Print and shaded views of the part. All mm, measured from the part's lowest x, y and z. Coordinates: 2 decimals unless noted, no trailing zeros. Order: outer loops, then holes, each group sorted by start corner. A loop starts at its lowest first (then second) coordinate and runs counter-clockwise, first axis right, second up. Notation, with made-up numbers: (22, -17) -> (54, -17) arc R26 ccw to (54, 20) -> close; hole circle Ø10 at (70.5, -2.75). An arc over 180 degrees is marked (long way). Write item = value, one per line. Start each with the question number.
Q1. Mould opens along Y. For the marked faces 1 and 2 say: +Y half, -Y half, draft (parallel to the pull), parting line (faces both ways), or undercut.
Q2. Flat gauge pins, fed straight in: pin 1 (8.5 mm diameter, centred on x = 82, y = 39, fed in from +Z); pin 2 (1.5 mm diameter, centred on y = 69.5, z = 6, fed in from -X) (1 decimal); pin 3 (4 mm diameter, centred on x = 81.5, z = 4.5, fed in from +Y); pin 4 (5 mm diameter, centred on x = 37, z = 4, fed in from -Y) (1 decimal). Where does each tip first touch, or does it go through?
Q3. Cut at B-B, the plane z = 1.75. List the corners of the cut face in (x, y), plus the area to 3 significant figures.
Q4. Cut at C-C, the plane y = 39. List the corners of the cut face in (x, z), plus the area to 3 significant figures.
Q5. Cut at A-A, the plane x = 82. List the corners of the cut face in (y, z), plus the area to 3 significant figures.
Q6. Cut at D-D, the plane y = 87.5. List the corners of the cut face in (x, z), plus the area to 3 significant figures.
Q7. Wall check: line 1 (Y direction, x = 82, z = 4.75); line 2 (X direction, y = 63.5, z = 7.75) (1 decimal); line 3 (X direction, y = 46.5, z = 6.5) (1 decimal). Give the ranges that are in metal, low to high. Write a range as from..to.
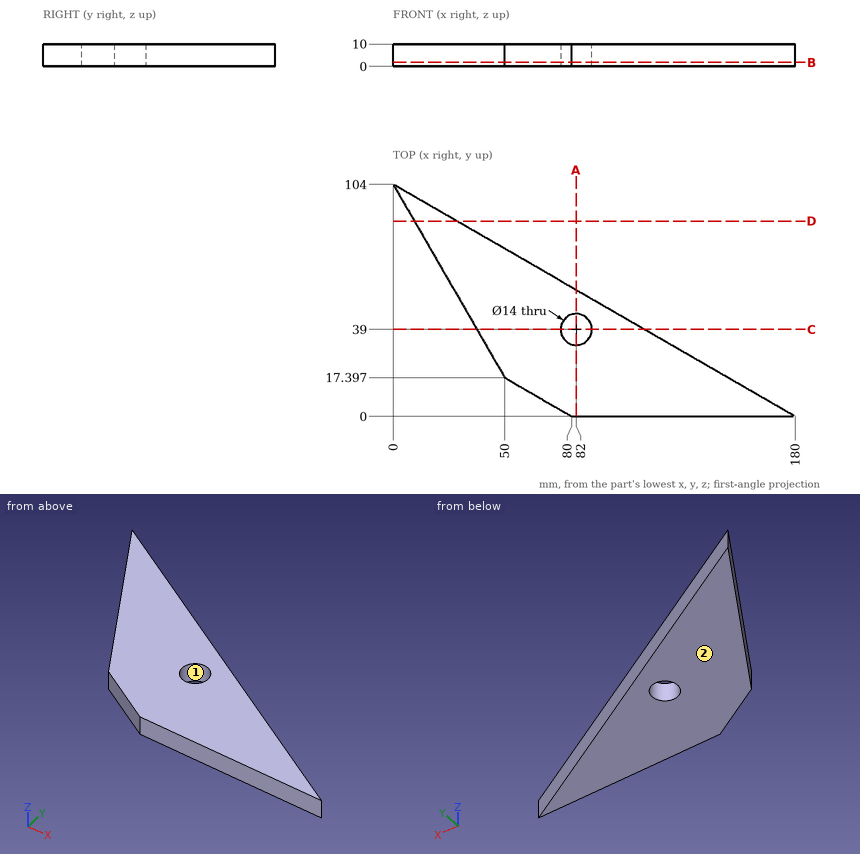
Here are the results:
q1.face_1 = undercut
q1.face_2 = draft
q2.pin_1 = through
q2.pin_2 = 19.5
q2.pin_3 = 58.07
q2.pin_4 = 35.6
q3.outline = (0, 104) -> (50, 17.4) -> (80, 0) -> (180, 0) -> close; hole circle Ø14 at (82, 39)
q3.area = 5,910 mm²
q4.outline = (37.53, 0) -> (75, 0) -> (75, 10) -> (37.53, 10) -> close; (89, 0) -> (112.5, 0) -> (112.5, 10) -> (89, 10) -> close
q4.area = 610 mm²
q5.outline = (0, 0) -> (32, 0) -> (32, 10) -> (0, 10) -> close; (46, 0) -> (56.62, 0) -> (56.62, 10) -> (46, 10) -> close
q5.area = 426 mm²
q6.outline = (9.53, 0) -> (28.56, 0) -> (28.56, 10) -> (9.53, 10) -> close
q6.area = 190 mm²
q7.line_1 = 0..32, 46..56.62
q7.line_2 = 23.4..70.1
q7.line_3 = 33.2..99.5
